Here's how the part is built. I have some questions about the finished solid (model axes, mm). Face numbers are marked on the shaded views. A direction names the side the tool comes from. Give positions to 0.01 mm unless a question says otherwise; leave off trailing zeros. Order: outer loops, then holes, each group sorted by start corner. A loop starts at its lowest first (then second) coordinate and runs counter-clockwise, first axis right, second up. Notation, with made-up numbers: (-28.75, 15) -> (-1.75, 15) arc R15 cw to (-1.75, 24) -> close; hole circle Ø1 at (68.25, 1). An arc over 180 degrees is marked (long way). Write each question's results on one line, items separated by ' | '. Start each with the question number.
Q1. Thinking about a two-plate mould opening in Y: for the marked faces 3, 4 and 5, which applies, pulls with the +Y half, pulls with the -Y half, needs draft (parallel to the pull), parting line crosses it, or undercut?
Q2. Imagine slicing it at C-C, the plane z = 4.25. Please give me the cut outline in (x, y).
Q3. For the marked faces 1 and 2, which set-ups out of +Z, -Z, +X, -X, +Y, -Y let a thin tool reach every point of the face, with its end or its side?
Q4. Imagine slicing it at A-A, the plane x = -7.5. Please give me the cut outline in (y, z).
Q5. Imagine slicing it at B-B, the plane y = 6. Please give me the cut outline in (x, z), then the cut area to 3 significant figures.
Q6. Imagine slicing it at D-D, the plane y = 1.5. Please give me the cut outline in (x, z).
Q7. I need wall thicknesses on line 1 along X through (y, z) = (5.75, 4.25); line 2 along X through (y, z) = (4.25, -2.5); line 3 along Y through (x, z) = (-7.5, -1.75). Which ranges of each line are inside material? Lowest first, please. Write a range as [from, to].
Q8. I'm going to push flat-ended pins straight in: pin 1 (5 mm diameter, centred on x = -7.5, y = 6, fed in from +Z); pin 2 (5 mm diameter, centred on x = 6.5, y = 4.5, fed in from -Z); pin 3 (5 mm diameter, centred on x = 8.5, y = 6, fed in from +Z). Where does each tip first touch, or does it pass through?
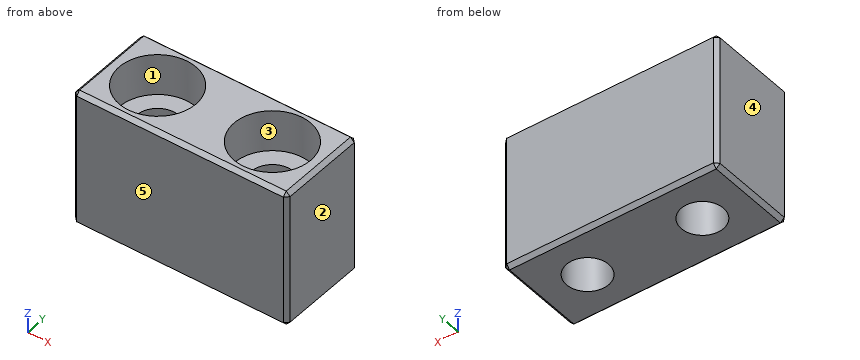
```python
from build123d import *

# Parameters (mm, degrees)
SKETCH_1_W                   = 28
SKETCH_1_H                   = 18
EXTRUDE_1_DEPTH              = 12
HOLE_WIZARD_M5_1_D           = 5.5
HOLE_WIZARD_M5_1_CBORE_D     = 10
HOLE_WIZARD_M5_1_CBORE_DEPTH = 5.4
CHAMFER_1_SIZE               = 0.5


with BuildPart() as part:
    # 草图1 → 凸台-拉伸1 (new body)
    with BuildSketch(Plane(origin=(0, 0, 0), x_dir=(1, 0, 0), z_dir=(0, 1, 0))):
        Rectangle(SKETCH_1_W, SKETCH_1_H)
    extrude(amount=EXTRUDE_1_DEPTH)

    # M5 六角凹头螺钉的柱形沉头孔1 (through all)
    with Locations(Plane.XY.offset(9)):
        with Locations((-7.5, 6), (7.5, 6)):
            CounterBoreHole(HOLE_WIZARD_M5_1_D / 2, HOLE_WIZARD_M5_1_CBORE_D / 2, HOLE_WIZARD_M5_1_CBORE_DEPTH)

    # 倒角1
    chamfer_1_edges = [part.edges().sort_by_distance(p)[0] for p in [
        (-14, 12, 0),
        (0, 12, 9),
        (14, 12, 0),
        (0, 0, 9),
        (-14, 0, 0),
        (0, 0, -9),
        (14, 0, 0),
        (0, 12, -9),
        (14, 6, 9),
        (-14, 6, 9),
        (-14, 6, -9),
        (14, 6, -9),
    ]]
    chamfer(chamfer_1_edges, length=CHAMFER_1_SIZE)


solid = part.part
```
Geometry check:
1) face 3: undercut | face 4: needs draft | face 5: pulls with the -Y half
2) outline: (-14, 0.5) -> (-13.5, 0) -> (13.5, 0) -> (14, 0.5) -> (14, 11.5) -> (13.5, 12) -> (-13.5, 12) -> (-14, 11.5) -> close; hole circle Ø10 at (-7.5, 6); hole circle Ø10 at (7.5, 6)
3) face 1: +Z | face 2: +Z, -Z, +X, +Y, -Y
4) outline: (0, -8.5) -> (0.5, -9) -> (3.25, -9) -> (3.25, 3.6) -> (1, 3.6) -> (1, 9) -> (0.5, 9) -> (0, 8.5) -> close; (8.75, -9) -> (11.5, -9) -> (12, -8.5) -> (12, 8.5) -> (11.5, 9) -> (11, 9) -> (11, 3.6) -> (8.75, 3.6) -> close
5) outline: (-14, -8.5) -> (-13.5, -9) -> (-10.25, -9) -> (-10.25, 3.6) -> (-12.5, 3.6) -> (-12.5, 9) -> (-13.5, 9) -> (-14, 8.5) -> close; (-4.75, -9) -> (4.75, -9) -> (4.75, 3.6) -> (2.5, 3.6) -> (2.5, 9) -> (-2.5, 9) -> (-2.5, 3.6) -> (-4.75, 3.6) -> close; (10.25, -9) -> (13.5, -9) -> (14, -8.5) -> (14, 8.5) -> (13.5, 9) -> (12.5, 9) -> (12.5, 3.6) -> (10.25, 3.6) -> close | area: 257 mm²
6) outline: (-14, -8.5) -> (-13.5, -9) -> (13.5, -9) -> (14, -8.5) -> (14, 8.5) -> (13.5, 9) -> (9.68, 9) -> (9.68, 3.6) -> (5.32, 3.6) -> (5.32, 9) -> (-5.32, 9) -> (-5.32, 3.6) -> (-9.68, 3.6) -> (-9.68, 9) -> (-13.5, 9) -> (-14, 8.5) -> close
7) line 1: [-14, -12.49], [-2.51, 2.51], [12.49, 14] | line 2: [-14, -9.62], [-5.38, 5.38], [9.62, 14] | line 3: [0, 3.25], [8.75, 12]
8) pin 1: through | pin 2: z = -9 | pin 3: z = 3.6
